Input: part model. Units: mm. Frame: model coordinates. A direction names the side the tool comes from. Give positions to 0.01 mm unless a question says otherwise; leave off trailing zeros. Write each loop counter-clockwise with the first axis right and the second up, starting at its lowest first coordinate (ties: lowest second). Pieces come first, ordered by that corner, then holes.
```python
from build123d import *

# Parameters (mm, degrees)
EXTRUDE_1_DEPTH     = 6.4
SKETCH_4_R          = 17.59
SKETCH_4_R_2        = 8
CUT_EXTRUDE_1_DEPTH = 0.8
CUT_EXTRUDE_1_DRAFT = -60
CHAMFER_1_SIZE      = 0.555555556


with BuildPart() as part:
    # 草图3 → 凸台-拉伸1 (new body)
    with BuildSketch(Plane(origin=(0, 0, 0), x_dir=(0, 0, -1), z_dir=(1, 0, 0))):
        Polygon((8, 4.618802154), (0, 9.237604307), (-8, 4.618802154), (-8, -4.618802154), (0, -9.237604307), (8, -4.618802154), align=None)
    extrude(amount=EXTRUDE_1_DEPTH)


with BuildPart() as cut_extrude_1_tool:
    # 草图4 → 切除-拉伸1 (with draft: the straight prism first)
    with BuildSketch(Plane.ZY):
        Circle(SKETCH_4_R)
        Circle(SKETCH_4_R_2, mode=Mode.SUBTRACT)
    extrude(amount=-CUT_EXTRUDE_1_DEPTH)
    # 切除-拉伸1: the draft: its side faces are tilted about the plane it starts from
    cut_extrude_1_sides = [cut_extrude_1_tool.faces().sort_by_distance(p)[0] for p in [
        (0.4, 0, -17.59),
        (0.4, 0, -8),
    ]]
    draft(cut_extrude_1_sides, Plane.ZY, CUT_EXTRUDE_1_DRAFT)


with BuildPart() as part_1:
    add(part.part)

    # 切除-拉伸1: cut by cut_extrude_1_tool
    add(cut_extrude_1_tool.part, mode=Mode.SUBTRACT)

    # 草图6 → 旋转2 (revolve)
    with BuildSketch(Plane.XY, mode=Mode.PRIVATE) as revolve_2_sk:
        with BuildLine():
            Line((10.9, 5), (41.4, 5))
            Line((41.4, 5), (41.4, 0))
            Line((41.4, 0), (6.4, 0))
            Line((6.4, 0), (6.4, 5.612875))
            ThreePointArc((6.4, 5.612875), (6.78085818, 4.780507868), (7.659700078, 4.524529519))
            Line((7.659700078, 4.524529519), (10.9, 5))
        make_face()
    revolve(revolve_2_sk.sketch.rotate(Axis((6.4, 0, 0), (1, 0, 0)), 180), axis=Axis((6.4, 0, 0), (1, 0, 0)))

    # 倒角1
    chamfer_1_edges = [part_1.edges().sort_by_distance(p)[0] for p in [
        (41.4, 5, 0),
    ]]
    chamfer(chamfer_1_edges, length=CHAMFER_1_SIZE)

    # 草图8 → 切除-旋转2 (revolve, cut)
    with BuildSketch(Plane.XY, mode=Mode.PRIVATE) as cut_revolve_2_sk:
        Polygon((6.4, 7.135), (5.8, 7.735), (5.8, 17.59), (6.4, 17.59), align=None)
    revolve(cut_revolve_2_sk.sketch.rotate(Axis((0, 0, 0), (1, 0, 0)), 180), axis=Axis((0, 0, 0), (1, 0, 0)), mode=Mode.SUBTRACT)


solid = part_1.part
```
Q1. Access query for faces 4 (the flat face through (0, 0, 0)), 5 (the flat face through (5.8, 3.38, -7.15)). Directions: +Z, -Z, +X, -X, +Y, -Y. A direction counts if a zero-diameter tool reaches every point of the face in a straight line with its end or side. Return the directions, or none.
Q2. Section A-A, the plane x = 38. Return the cut outline in (y, z).
Q3. Material intervals for line 1 along Z through (x, y) = (12, 0); line 2 along X through (y, z) = (5, 4); line 3 along Z through (x, y) = (6, -4), sorted ascending.
Q4. Mould query, pull axis X, two halves, no side actions, for faces 1 (the conical face through (8.58, 0.61, -4.62)), 2 (the flat face through (3, 0, 8)), 3 (the conical face through (0.17, -8.295, -0.02)). Classes: +X half, -X half, draft (parallel to the pull), parting line (faces both ways), or undercut.
Q5. Pin query (flat end, axial travel): pin 1 (5 mm diameter, centred on x = 29, y = -3.5, fed in from -Z); pin 2 (10 mm diameter, centred on x = 35.5, y = -7, fed in from +Z); pin 3 (3 mm diameter, centred on x = 32, z = 2.5, fed in from +Y). Return the tip coordinate at first contact, or that it passes through.
Solutions:
1. face 4: +Z, -Z, -X, +Y, -Y
1. face 5: +X
2. outline: circle Ø10 at (0, 0)
3. line 1: z = -5 to 5
3. line 2: x = 0 to 6.4
3. line 3: z = -6.39 to 6.39
4. face 1: undercut
4. face 2: draft
4. face 3: -X half
5. pin 1: stops at z = -4.9
5. pin 2: stops at z = 4.58
5. pin 3: stops at y = 4.9
